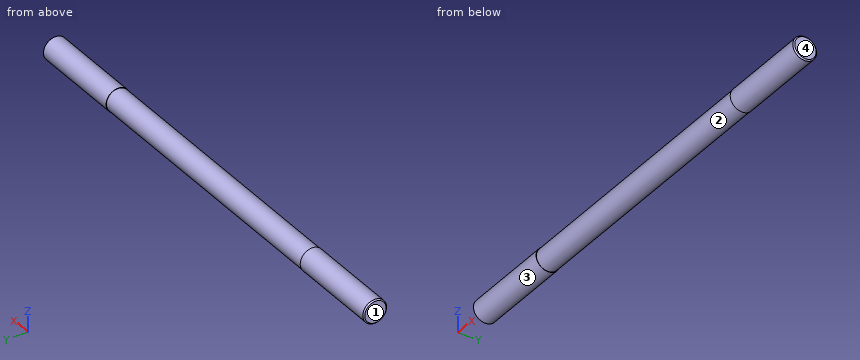
```python
from build123d import *

# Parameters (mm, degrees)
CHAMFER1_SIZE = 1


with BuildPart() as part:
    # Sketch3 → Revolve1 (revolve)
    with BuildSketch(Plane.XY, mode=Mode.PRIVATE) as revolve1_sk:
        Polygon((325, 10), (405, 10), (405, 0), (0, 0), (0, 10), (80, 10), (80, 9.75), (325, 9.75), align=None)
    revolve(revolve1_sk.sketch.rotate(Axis((0, 0, 0), (1, 0, 0)), 90), axis=Axis((0, 0, 0), (1, 0, 0)))

    # Chamfer1
    chamfer1_edges = [part.edges().sort_by_distance(p)[0] for p in [
        (405, 0, -10),
        (0, 0, -10),
    ]]
    chamfer(chamfer1_edges, length=CHAMFER1_SIZE)


solid = part.part
```
Can you work these out from the model? Positions are in its coordinate system, mm. Face numbers are marked on the shaded views. Round coordinates to 2 decimals unless told otherwise and drop trailing zeros. Loops run counter-clockwise (first coordinate to the right, second up) from the corner with the lowest first, then second, coordinate; pieces in that order, holes last. Notation, with made-up numbers: (12, 87.25) -> (44, 87.25) arc R14 ccw to (44, 114.25) -> close; hole circle Ø9 at (65, 18.5). An arc over 180 degrees is marked (long way). One line per item, written item: value. Start each with the question number.
1. If we section it at A-A, the plane z = 0: Write out the boundary of the cut face in (x, y), then the cut area to 3 significant figures.
2. If I drill on probe 1 along Y at (x, z) = (125.5, -0.75); probe 2 along Y at (x, z) = (357, -0.5); probe 3 along X at (y, z) = (-5.5, 8.25), over which ranges is the centre line in solid material (lowest first)?
3. For pin 1 (12 mm diameter, centred on y = 2.5, z = 0, fed in from -X); pin 2 (8 mm diameter, centred on x = 129.5, y = 2, fed in from +Z); pin 3 (10 mm diameter, centred on x = 118.5, z = 6.5, fed in from -Y); pin 4 (12 mm diameter, centred on x = 106.5, z = -0.5, fed in from -Y), each with a flat end and sliding along its axis, tell me the tip position at first contact or that it passes through.
4. If we mould it in two halves opening along X, with no side actions, what happens to the marked faces 1, 2, 3 and 4? For each: pulls with the +X half, pulls with the -X half, needs draft (parallel to the pull), parting line crosses it, or undercut.
5. If we section it at C-C, the plane x = 336: Write out the boundary of the cut face in (y, z).
Calculated:
1. outline: (0, -9) -> (1, -10) -> (80, -10) -> (80, -9.75) -> (325, -9.75) -> (325, -10) -> (404, -10) -> (405, -9) -> (405, 9) -> (404, 10) -> (325, 10) -> (325, 9.75) -> (80, 9.75) -> (80, 10) -> (1, 10) -> (0, 9) -> close
1. area: 7,980 mm²
2. probe 1: y = -9.72 to 9.72
2. probe 2: y = -9.99 to 9.99
2. probe 3: x = 0.92 to 80, 325 to 404.08
3. pin 1: stops at x = 0
3. pin 2: stops at z = 9.75
3. pin 3: stops at y = -9.63
3. pin 4: stops at y = -9.75
4. face 1: pulls with the -X half
4. face 2: undercut
4. face 3: needs draft
4. face 4: pulls with the +X half
5. outline: circle Ø20 at (0, 0)
